```python
from build123d import *

# Parameters (mm, degrees)
SKETCH1_W           = 2000
SKETCH1_H           = 2160
BOSS_EXTRUDE1_DEPTH = 30
SKETCH2_R           = 10
BOSS_EXTRUDE2_DEPTH = 50
SKETCH3_R           = 32
CUT_EXTRUDE1_DEPTH  = 40


with BuildPart() as part:
    # Sketch1 → Boss-Extrude1 (new body)
    with BuildSketch(Plane(origin=(0, 0, 0), x_dir=(1, 0, 0), z_dir=(0, 1, 0))):
        Rectangle(SKETCH1_W, SKETCH1_H)
    extrude(amount=BOSS_EXTRUDE1_DEPTH)

    # Sketch2 → Boss-Extrude2 (add)
    with BuildSketch(Plane(origin=(0, 30, 0), x_dir=(1, 0, 0), z_dir=(0, 1, 0))):
        with Locations(Location((-920, 1000, 0), (0, 0, 90))):
            Circle(SKETCH2_R)
        with Locations(Location((-920, 760, 0), (0, 0, 90))):
            Circle(SKETCH2_R)
        with Locations(Location((-480, 1000, 0), (0, 0, 90))):
            Circle(SKETCH2_R)
        with Locations(Location((-480, 760, 0), (0, 0, 90))):
            Circle(SKETCH2_R)
        with Locations(Location((480, 760, 0), (0, 0, 90))):
            Circle(SKETCH2_R)
        with Locations(Location((480, 1000, 0), (0, 0, 90))):
            Circle(SKETCH2_R)
        with Locations(Location((920, 760, 0), (0, 0, 90))):
            Circle(SKETCH2_R)
        with Locations(Location((920, 1000, 0), (0, 0, 90))):
            Circle(SKETCH2_R)
        with Locations(Location((920, -1000, 0), (0, 0, 90))):
            Circle(SKETCH2_R)
        with Locations(Location((920, -760, 0), (0, 0, 90))):
            Circle(SKETCH2_R)
        with Locations(Location((480, -1000, 0), (0, 0, 90))):
            Circle(SKETCH2_R)
        with Locations(Location((480, -760, 0), (0, 0, 90))):
            Circle(SKETCH2_R)
        with Locations(Location((-480, -760, 0), (0, 0, 90))):
            Circle(SKETCH2_R)
        with Locations(Location((-480, -1000, 0), (0, 0, 90))):
            Circle(SKETCH2_R)
        with Locations(Location((-920, -760, 0), (0, 0, 90))):
            Circle(SKETCH2_R)
        with Locations(Location((-920, -1000, 0), (0, 0, 90))):
            Circle(SKETCH2_R)
    extrude(amount=BOSS_EXTRUDE2_DEPTH)

    # Sketch3 → Cut-Extrude1 (cut)
    with BuildSketch(Plane(origin=(0, 30, 0), x_dir=(1, 0, 0), z_dir=(0, 1, 0))):
        with Locations(Location((0, 880, 0), (0, 0, 270))):
            Circle(SKETCH3_R)
        with Locations(Location((0, -880, 0), (0, 0, 270))):
            Circle(SKETCH3_R)
    extrude(amount=-CUT_EXTRUDE1_DEPTH, mode=Mode.SUBTRACT)


solid = part.part
```
Could you check a few things on this model? Use its own coordinates, in mm. Round coordinates to 2 decimals unless told otherwise and drop trailing zeros. Write each loop counter-clockwise with the first axis right and the second up, starting at its lowest first coordinate (ties: lowest second). Pieces come first, ordered by that corner, then holes. Notation, with made-up numbers: M 86.25,21 L 104.25,21 A35 cw 104.25,56 Z; hole C 4.25,66.5 d1. An arc over 180 degrees is marked long. Answer in a Markdown table with one row per item. Add a question column.
Q1. Imagine slicing it at C-C (z = 198.5). Please give me the cut outline in (x, y).
Q2. Will this pin go through, and if not, where does the flat tip stop? pin 1 Ø10 at (x, z) = (-18, -681) entering from +Y.
Q3. Imagine slicing it at B-B (z = -880). Please give me the cut outline in (x, y).
Q4. If we mould it in two halves opening along Z, with no side actions, what happens to faces 1 (the flat face through (-14, 0, -15)), 2 (the cylindrical face through (1.41, 15.21, -911.97))? For each: +Z half, -Z half, draft (parallel to the pull), parting line (faces both ways), or undercut.
Q5. Imagine slicing it at A-A (x = 0). Please give me the cut outline in (y, z), then the cut area to 3 significant figures.
Q6. If I drill on line 1 (X direction, y = 19.75, z = -880); line 2 (Y direction, x = 396, z = -958.5), over which ranges is the centre line in solid material (lowest first)? Write a range as from..to.
Values:
| question | item | result |
|---|---|---|
| 1 | outline | M -1000,0 L 1000,0 L 1000,30 L -1000,30 Z |
| 2 | pin 1 | y = 30 |
| 3 | outline | M -1000,0 L -32,0 L -32,30 L -1000,30 Z; M 32,0 L 1000,0 L 1000,30 L 32,30 Z |
| 4 | face 1 | draft |
| 4 | face 2 | undercut |
| 5 | outline | M 0,-1080 L 30,-1080 L 30,-912 L 0,-912 Z; M 0,-848 L 30,-848 L 30,848 L 0,848 Z; M 0,912 L 30,912 L 30,1080 L 0,1080 Z |
| 5 | area | 61,000 mm^2 |
| 6 | line 1 | -1000..-32, 32..1000 |
| 6 | line 2 | 0..30 |
